Model file for the job. Use its own axes, mm. Face numbers are marked on the shaded views. A direction names the side the tool comes from. Coordinates: 2 decimals unless noted, no trailing zeros. Order: outer loops, then holes, each group sorted by start corner. A loop starts at its lowest first (then second) coordinate and runs counter-clockwise, first axis right, second up. Notation, with made-up numbers: (47.25, -15) -> (51.25, -15) arc R18 cw to (51.25, -1) -> close; hole circle Ø8 at (43.25, -31). An arc over 180 degrees is marked (long way). Use CSV: the item, a comma, the result in double quotes. Start each with the question number.
(1) Pin check, flat tips, straight feed: pin 1 Ø1 at (x, z) = (14, -1.5) entering from -Y; pin 2 Ø1.2 at (y, z) = (-0.5, 2) entering from +X; pin 3 Ø1 at (x, z) = (0, -3) entering from -Y. Stop position of each tip, or through.
(2) Tool access for the marked faces 4, 5 and 6: list every direction of +Z, -Z, +X, -X, +Y, -Y with a clear straight run to the whole face (end or side of a thin tool).
(3) Cut at D-D on z = 0.75. Write the cut outline in (x, y).
(4) Probe L1, parallel to Y at x = 0, z = -3.75; L2, parallel to Z at x = 0, y = -10.5; L3, parallel to X at y = -3.25, z = -4.5. List the from-to ranges inside material, lowest first.
(5) Cut at A-A on x = 0. Write the cut outline in (y, z), plus the area to 3 significant figures.
(6) Pull direction Z, two halves, no side cores. Call the marked faces 1, 2 and 3: pulls with the +Z half, pulls with the -Z half, needs draft (parallel to the pull), parting line crosses it, or undercut.
(7) Cut at B-B on z = 4. Write the cut outline in (x, y).
(8) Cut at C-C on y = 0. Write the cut outline in (x, z).
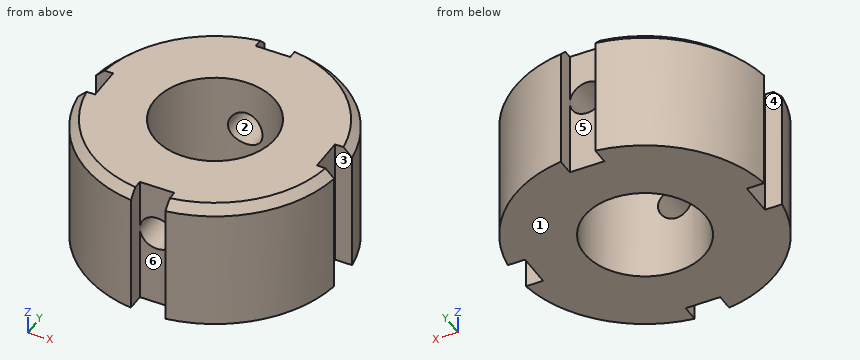
```python
from build123d import *

# Parameters (mm, degrees)
NUT_BODY_15MM_DEPTH       = 7.5
M16_TAPPED_THROUGH_HOLE_D = 14
EDGE_CHAMFER_1X45_SIZE    = 1
CROSS_HOLE_4_DEPTH        = 23.321514286
CROSS_HOLE_4_DEPTH_BACK   = 23.321514286
CROSS_HOLE_4_SKETCH_R     = 2


with BuildPart() as part:
    # Slotted Nut Profile Ø30 → Nut Body 15mm (new, symmetric)
    with BuildSketch(Plane.XY):
        with BuildLine():
            Line((2, 12.866068747), (2, 14.866068747))
            ThreePointArc((2, 14.866068747), (10.606601718, 10.606601718), (14.866068747, 2))
            Line((14.866068747, 2), (12.866068747, 2))
            Line((12.866068747, 2), (12.866068747, -2))
            Line((12.866068747, -2), (14.866068747, -2))
            ThreePointArc((14.866068747, -2), (10.606601718, -10.606601718), (2, -14.866068747))
            Line((2, -14.866068747), (2, -12.866068747))
            Line((2, -12.866068747), (-2, -12.866068747))
            Line((-2, -12.866068747), (-2, -14.866068747))
            ThreePointArc((-2, -14.866068747), (-10.606601718, -10.606601718), (-14.866068747, -2))
            Line((-14.866068747, -2), (-12.866068747, -2))
            Line((-12.866068747, -2), (-12.866068747, 2))
            Line((-12.866068747, 2), (-14.866068747, 2))
            ThreePointArc((-14.866068747, 2), (-10.606601718, 10.606601718), (-2, 14.866068747))
            Line((-2, 14.866068747), (-2, 12.866068747))
            Line((-2, 12.866068747), (2, 12.866068747))
        make_face()
    extrude(amount=NUT_BODY_15MM_DEPTH, both=True)

    # M16 Tapped Through Hole (through all)
    with Locations(Plane.XY.offset(7.5)):
        with Locations((0, 0)):
            Hole(M16_TAPPED_THROUGH_HOLE_D / 2)

    # Edge Chamfer 1x45°
    edge_chamfer_1x45_edges = [part.edges().sort_by_distance(p)[0] for p in [
        (-10.606601718, 10.606601718, 7.5),
        (-10.606601718, -10.606601718, 7.5),
        (10.606601718, -10.606601718, 7.5),
        (10.606601718, 10.606601718, 7.5),
    ]]
    chamfer(edge_chamfer_1x45_edges, length=EDGE_CHAMFER_1X45_SIZE)

    # Cross Hole Ø4 Sketch → Cross Hole Ø4 (cut, two sides: drawn at the far end of the back side and taken through both)
    with BuildSketch(Plane(origin=(0, 0, 0), x_dir=(1, 0, 0), z_dir=(0, 1, 0)).offset(-CROSS_HOLE_4_DEPTH_BACK)):
        with Locations(Location((0, -1.5, 0), (0, 0, 270))):
            Circle(CROSS_HOLE_4_SKETCH_R)
    extrude(amount=CROSS_HOLE_4_DEPTH + CROSS_HOLE_4_DEPTH_BACK, mode=Mode.SUBTRACT)


solid = part.part
```
Outcome:
1,pin 1,"y = -6.54"
1,pin 2,"x = 12.87"
1,pin 3,"y = -12.87"
2,face 4,"+Z, -Z, -X"
2,face 5,"+Z, -Z, +Y"
2,face 6,"+Z, -Z, -Y"
3,outline,"(-14.87, -2) arc R15 ccw to (-2, -14.87) -> (-2, -12.87) -> (-1.85, -12.87) -> (-1.85, -6.75) arc R7 cw to (-1.85, 6.75) -> (-1.85, 12.87) -> (-2, 12.87) -> (-2, 14.87) arc R15 ccw to (-14.87, 2) -> (-12.87, 2) -> (-12.87, -2) -> close; (1.85, -12.87) -> (2, -12.87) -> (2, -14.87) arc R15 ccw to (14.87, -2) -> (12.87, -2) -> (12.87, 2) -> (14.87, 2) arc R15 ccw to (2, 14.87) -> (2, 12.87) -> (1.85, 12.87) -> (1.85, 6.75) arc R7 cw to (1.85, -6.75) -> close"
4,L1,"-12.87 to -7, 7 to 12.87"
4,L2,"-7.5 to -0.5, 3.5 to 7.5"
4,L3,"-14.64 to -6.2, 6.2 to 14.64"
5,outline,"(-12.87, -7.5) -> (-7, -7.5) -> (-7, -0.5) -> (-12.87, -0.5) -> close; (-12.87, 3.5) -> (-7, 3.5) -> (-7, 7.5) -> (-12.87, 7.5) -> close; (7, -7.5) -> (12.87, -7.5) -> (12.87, -0.5) -> (7, -0.5) -> close; (7, 3.5) -> (12.87, 3.5) -> (12.87, 7.5) -> (7, 7.5) -> close"
5,area,"129 mm2"
6,face 1,"pulls with the -Z half"
6,face 2,"undercut"
6,face 3,"needs draft"
7,outline,"(-14.87, -2) arc R15 ccw to (-2, -14.87) -> (-2, -12.87) -> (2, -12.87) -> (2, -14.87) arc R15 ccw to (14.87, -2) -> (12.87, -2) -> (12.87, 2) -> (14.87, 2) arc R15 ccw to (2, 14.87) -> (2, 12.87) -> (-2, 12.87) -> (-2, 14.87) arc R15 ccw to (-14.87, 2) -> (-12.87, 2) -> (-12.87, -2) -> close; hole circle Ø14 at (0, 0)"
8,outline,"(-12.87, -7.5) -> (-7, -7.5) -> (-7, 7.5) -> (-12.87, 7.5) -> close; (7, -7.5) -> (12.87, -7.5) -> (12.87, 7.5) -> (7, 7.5) -> close"
